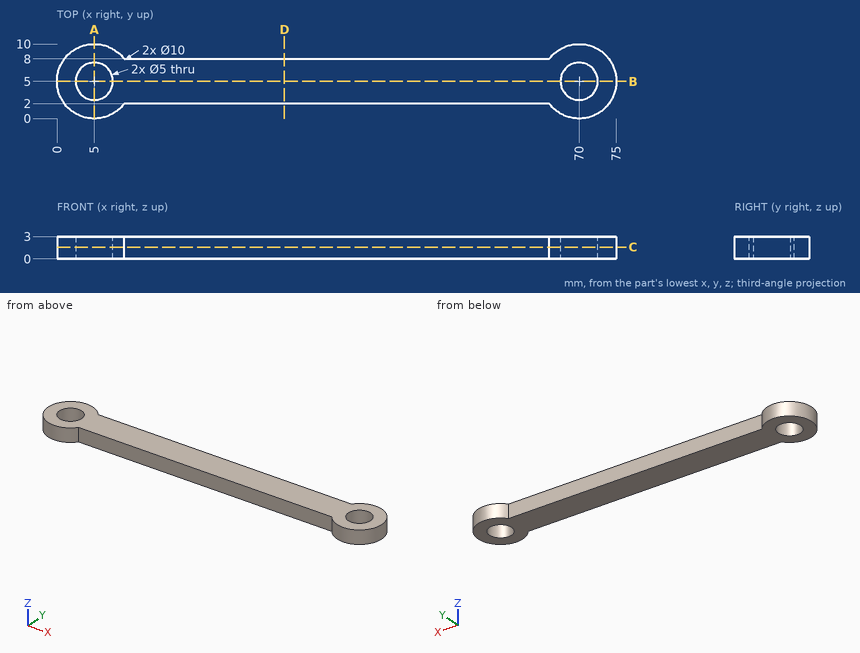
The drawing under review shows one solid part. Ordinate dimensions are in mm from its lowest x, y, z. Give positions to 0.01 mm unless a question says otherwise; leave off trailing zeros. Order: outer loops, then holes, each group sorted by start corner. A loop starts at its lowest first (then second) coordinate and runs counter-clockwise, first axis right, second up. Notation, with made-up numbers: (45, -9) -> (49, -9) arc R15 cw to (49, 3) -> close; hole circle Ø3 at (-32, 14). An arc over 180 degrees is marked (long way). Write item = value, one per line. Start each with the question number.
(1) To check wall thickness, follow line 1 along X through (y, z) = (4.75, 2.65); line 2 along X through (y, z) = (4.25, 1.4); line 3 along Y through (x, z) = (70, 0.9). State the ranges of each line that lie inside material, in increasing order.
(2) We need section B-B on y = 5. Write out the cut boundary in (x, z), plus the area to 3 significant figures.
(3) For pin 1 (0.9 mm diameter, centred on x = 32.5, z = 1.5, fed in from -Y); pin 2 (0.9 mm diameter, centred on x = 30, z = 1.5, fed in from +Y), all flat-tipped, find the tip position at first contact; note any pin that passes through.
(4) We need section A-A on x = 5. Write out the cut boundary in (y, z), plus the area to 3 significant figures.
(5) We need section D-D on x = 30.5. Write out the cut boundary in (y, z), plus the area to 3 significant figures.
(6) We need section C-C on z = 1.6. Write out the cut boundary in (x, y).
Numbers:
q1.line_1 = 0.01 to 2.51, 7.49 to 67.51, 72.49 to 74.99
q1.line_2 = 0.06 to 2.62, 7.38 to 67.62, 72.38 to 74.94
q1.line_3 = 0 to 2.5, 7.5 to 10
q2.outline = (0, 0) -> (2.5, 0) -> (2.5, 3) -> (0, 3) -> close; (7.5, 0) -> (67.5, 0) -> (67.5, 3) -> (7.5, 3) -> close; (72.5, 0) -> (75, 0) -> (75, 3) -> (72.5, 3) -> close
q2.area = 195 mm^2
q3.pin_1 = 2
q3.pin_2 = 8
q4.outline = (0, 0) -> (2.5, 0) -> (2.5, 3) -> (0, 3) -> close; (7.5, 0) -> (10, 0) -> (10, 3) -> (7.5, 3) -> close
q4.area = 15.0 mm^2
q5.outline = (2, 0) -> (8, 0) -> (8, 3) -> (2, 3) -> close
q5.area = 18.0 mm^2
q6.outline = (9, 2) -> (66, 2) arc R5 ccw (long way) to (66, 8) -> (9, 8) arc R5 ccw (long way) to start; hole circle Ø5 at (5, 5); hole circle Ø5 at (70, 5)
